from build123d import *

# Parameters (mm, degrees)
BOSS_EXTRUDE1_DEPTH = 3


with BuildPart() as part:
    # Sketch1 → Boss-Extrude1 (new body)
    with BuildSketch(Plane.XY):
        with BuildLine():
            Line((0, 5), (0, 415))
            ThreePointArc((0, 415), (1.464466094, 418.535533906), (5, 420))
            Line((5, 420), (273.602650759, 420))
            ThreePointArc((273.602650759, 420), (275.794506493, 419.493970231), (277.542704528, 418.078307377))
            Line((277.542704528, 418.078307377), (396.940053768, 265.25666931))
            ThreePointArc((396.940053768, 265.25666931), (397.727592878, 263.806202706), (398, 262.178361934))
            Line((398, 262.178361934), (398, 5))
            ThreePointArc((398, 5), (396.535533906, 1.464466094), (393, 0))
            Line((393, 0), (289, 0))
            Line((289, 0), (289, 90))
            ThreePointArc((289, 90), (199, 180), (109, 90))
            Line((109, 90), (109, 0))
            Line((109, 0), (5, 0))
            ThreePointArc((5, 0), (1.464466094, 1.464466094), (0, 5))
        make_face()
    extrude(amount=BOSS_EXTRUDE1_DEPTH)


solid = part.part
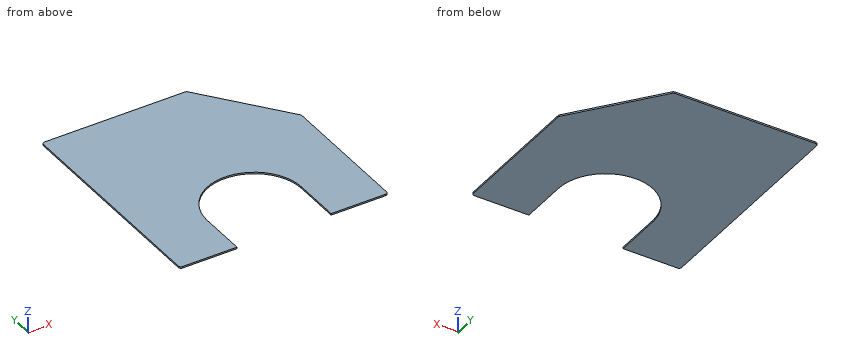
Read the model definition and answer for the solid it produces. Units are mm, in the model's axes. Coordinates: 2 decimals unless noted, no trailing zeros. Write each loop counter-clockwise with the first axis right and the second up, starting at its lowest first coordinate (ties: lowest second). Pieces come first, ordered by that corner, then holes. Notation, with made-up numbers: (29, 62) -> (72, 62) arc R11 ccw to (72, 82) -> close; hole circle Ø10 at (21.25, 3.5). An arc over 180 degrees is marked (long way). Return JSON: item names as keys, results as strings.
(1) The part is cut by section B-B on z = 0.9. Give the vertices of the cut face in (x, y).
Answers below:
{"outline": "(0, 5) arc R5 ccw to (5, 0) -> (109, 0) -> (109, 90) arc R90 cw to (289, 90) -> (289, 0) -> (393, 0) arc R5 ccw to (398, 5) -> (398, 262.18) arc R5 ccw to (396.94, 265.26) -> (277.54, 418.08) arc R5 ccw to (273.6, 420) -> (5, 420) arc R5 ccw to (0, 415) -> close"}
(2) The part is cut by section A-A on y = 62.5. Give the vertices of the cut face in (x, z), then the cut area to 3 significant figures.
Answers below:
{"outline": "(0, 0) -> (109, 0) -> (109, 3) -> (0, 3) -> close; (289, 0) -> (398, 0) -> (398, 3) -> (289, 3) -> close", "area": "654 mm^2"}
(3) Consider line 1 along X through (y, z) = (37, 1.3); line 2 along Y through (x, z) = (140, 2); line 3 along X through (y, z) = (276.5, 0.95). Determine where each line is inside the solid, lowest interval first. Write a range as from..to.
Answers below:
{"line 1": "0..109, 289..398", "line 2": "157.96..420", "line 3": "0..388.16"}
(4) The part is cut by section D-D on y = 108.5. Give the vertices of the cut face in (x, z).
Answers below:
{"outline": "(0, 0) -> (110.92, 0) -> (110.92, 3) -> (0, 3) -> close; (287.08, 0) -> (398, 0) -> (398, 3) -> (287.08, 3) -> close"}
(5) The part is cut by section C-C on x = 199. Give the vertices of the cut face in (y, z).
Answers below:
{"outline": "(180, 0) -> (420, 0) -> (420, 3) -> (180, 3) -> close"}
